from build123d import *

# Parameters (mm, degrees)
SKETCH_1_R          = 30
EXTRUDE_1_DEPTH     = 1300
SKETCH_2_R          = 24
CUT_EXTRUDE_1_DEPTH = 1600
SKETCH_3_R          = 26
CUT_EXTRUDE_2_DEPTH = 15
CUT_EXTRUDE_START   = -15
SKETCH_4_R          = 26
CUT_EXTRUDE_3_DEPTH = 15
CHAMFER_1_SIZE      = 0.5


with BuildPart() as part:
    # 草图1 → 凸台-拉伸1 (new body)
    with BuildSketch(Plane.XY):
        Circle(SKETCH_1_R)
    extrude(amount=EXTRUDE_1_DEPTH)

    # 草图2 → 切除-拉伸1 (cut)
    with BuildSketch(Plane(origin=(0, 0, 0), x_dir=(-1, 0, 0), z_dir=(0, 0, -1))):
        Circle(SKETCH_2_R)
    extrude(amount=-CUT_EXTRUDE_1_DEPTH, mode=Mode.SUBTRACT)

    # 草图3 → 切除-拉伸2 (cut)
    with BuildSketch(Plane(origin=(0, 0, 0), x_dir=(-1, 0, 0), z_dir=(0, 0, -1))):
        Circle(SKETCH_3_R)
    extrude(amount=-CUT_EXTRUDE_2_DEPTH, mode=Mode.SUBTRACT)

    # 草图4 → 切除-拉伸3 (cut)
    with BuildSketch(Plane.XY.offset(1300).offset(CUT_EXTRUDE_START)):
        with Locations(Location((0, 0, 0), (0, 0, 180))):
            Circle(SKETCH_4_R)
    extrude(amount=CUT_EXTRUDE_3_DEPTH, mode=Mode.SUBTRACT)

    # 倒角1
    chamfer_1_edges = [part.edges().sort_by_distance(p)[0] for p in [
        (26, 0, 0),
        (-30, 0, 0),
        (26, 0, 1300),
        (-30, 0, 1300),
    ]]
    chamfer(chamfer_1_edges, length=CHAMFER_1_SIZE)


solid = part.part
Can you work these out from the model? Positions are in its coordinate system, mm. A direction names the side the tool comes from. Coordinates: 2 decimals unless noted, no trailing zeros. Order: outer loops, then holes, each group sorted by start corner. A loop starts at its lowest first (then second) coordinate and runs counter-clockwise, first axis right, second up. Notation, with made-up numbers: M 63,-9 L 73,-9 A20 ccw 73,18 Z; hole C -31.75,-27.75 d11. An arc over 180 degrees is marked long. Write item = value, one per line.
(1) I need wall thicknesses on line 1 along Y through (x, z) = (0, 1293.25); line 2 along Y through (x, z) = (1.5, 1187.5); line 3 along X through (y, z) = (-2, 768.5). Which ranges of each line are inside material? Lowest first, please. Write a range as [from, to].
Results are:
line_1 = [-30, -26], [26, 30]
line_2 = [-29.96, -23.95], [23.95, 29.96]
line_3 = [-29.93, -23.92], [23.92, 29.93]
(2) Suppose I cut it at C-C on z = 123.5. Please give me the cut outline in (x, y), plus the area to 3 significant figures.
Results are:
outline = C 0,0 d60; hole C 0,0 d48
area = 1,020 mm2
(3) For faces 1 (the face through (-8, 23, 1285)), 2 (the face through (-8, -23, 15)), 3 (the face through (23.977, 1.055, 641.11)), which set-ups out of +Z, -Z, +X, -X, +Y, -Y let a thin tool reach every point of the face, with its end or its side?
Results are:
face_1 = +Z
face_2 = -Z
face_3 = +Z, -Z
(4) For pin 1 Ø5 at (x, z) = (-19.5, 1164) entering from +Y; pin 2 Ø6 at (y, z) = (-10.5, 323) entering from -X; pin 3 Ø1.5 at (x, z) = (11.5, 618) entering from -Y; pin 4 Ø8 at (x, y) = (5.5, -18) entering from +Z, each with a flat end and sliding along its axis, tell me the tip position at first contact or that it passes through.
Results are:
pin_1 = 24.72
pin_2 = -29.05
pin_3 = -28.01
pin_4 = through
(5) Suppose I cut it at A-A on y = 0. Please give me the cut outline in (x, z), plus the area to 3 significant figures.
Results are:
outline = M -30,0.5 L -29.5,0 L -26.5,0 L -26,0.5 L -26,15 L -24,15 L -24,1285 L -26,1285 L -26,1299.5 L -26.5,1300 L -29.5,1300 L -30,1299.5 Z; M 24,15 L 26,15 L 26,0.5 L 26.5,0 L 29.5,0 L 30,0.5 L 30,1299.5 L 29.5,1300 L 26.5,1300 L 26,1299.5 L 26,1285 L 24,1285 Z
area = 15,500 mm2
(6) If we mould it in two halves opening along X, with no side actions, what happens to faces 4 (the face through (-29.97, 1.32, 640.91)), 5 (the face through (20.633, -15.821, 7.648)), 6 (the face through (-20, 18, 0))? For each: pulls with the +X half, pulls with the -X half, needs draft (parallel to the pull), parting line crosses it, or undercut.
Results are:
face_4 = parting line crosses it
face_5 = undercut
face_6 = needs draft
